from build123d import *

# Parameters (mm, degrees)
SKETCH_1_W          = 365
SKETCH_1_H          = 55
EXTRUDE_1_DEPTH     = 12
SKETCH_2_R          = 10
CUT_EXTRUDE_1_DEPTH = 2
SKETCH_3_W          = 12
SKETCH_3_H          = 55
CUT_EXTRUDE_2_DEPTH = 1.5


with BuildPart() as part:
    # 草图1 → 凸台-拉伸1 (new body)
    with BuildSketch(Plane.XY):
        Rectangle(SKETCH_1_W, SKETCH_1_H)
    extrude(amount=EXTRUDE_1_DEPTH)

    # 草图2 → 切除-拉伸1 (cut)
    with BuildSketch(Plane.XY.offset(12)):
        with Locations((85, 0)):
            Circle(SKETCH_2_R)
        with Locations((-85, 0)):
            Circle(SKETCH_2_R)
    extrude(amount=-CUT_EXTRUDE_1_DEPTH, mode=Mode.SUBTRACT)

    # 草图3 → 切除-拉伸2 (cut)
    with BuildSketch(Plane(origin=(0, 0, 0), x_dir=(-1, 0, 0), z_dir=(0, 0, -1))):
        with Locations((176.5, 0)):
            Rectangle(SKETCH_3_W, SKETCH_3_H)
        with Locations((-176.5, 0)):
            Rectangle(SKETCH_3_W, SKETCH_3_H)
    extrude(amount=-CUT_EXTRUDE_2_DEPTH, mode=Mode.SUBTRACT)


solid = part.part
Source: CAD feature listing. Evaluate the final solid. Frame: model axes, mm. A direction names the side the tool comes from. Coordinates: 2 decimals unless noted, no trailing zeros. Write each loop counter-clockwise with the first axis right and the second up, starting at its lowest first coordinate (ties: lowest second). Pieces come first, ordered by that corner, then holes. Notation, with made-up numbers: M -21,-22.5 L 8,-22.5 A23 cw 8,-7.5 Z; hole C 33,0.25 d11. An arc over 180 degrees is marked long. Use a Markdown table: item, result.
1) Reachability of faces 4 (the flat face through (85, 0, 10)), 5 (the flat face through (-3, -27.5, 6)), 6 (the flat face through (177, 0, 1.5)) from +Z, -Z, +X, -X, +Y, -Y: full face, straight path, thin tool, end or side. Return the list, or none.
Conclusion:
| item | result |
|---|---|
| face 4 | +Z |
| face 5 | +Z, -Z, +X, -X, -Y |
| face 6 | -Z, +X, +Y, -Y |
2) First-contact query: pin 1 Ø10 at (x, y) = (-87, -2) entering from +Z; pin 2 Ø6 at (x, y) = (-178, -8.5) entering from -Z; pin 3 Ø1.2 at (y, z) = (3.5, 0.5) entering from +X. Flat tips, straight axial feed; report the tip coordinate or a pass-through.
Conclusion:
| item | result |
|---|---|
| pin 1 | stops at z = 10 |
| pin 2 | stops at z = 1.5 |
| pin 3 | stops at x = 170.5 |
3) Section A-A, the plane y = 0. Output: boundary loops of the cut face in (x, z).
Conclusion:
| item | result |
|---|---|
| outline | M -182.5,1.5 L -170.5,1.5 L -170.5,0 L 170.5,0 L 170.5,1.5 L 182.5,1.5 L 182.5,12 L 95,12 L 95,10 L 75,10 L 75,12 L -75,12 L -75,10 L -95,10 L -95,12 L -182.5,12 Z |
4) Ray query, L1, parallel to Y at x = -85, z = 11.45; L2, parallel to Z at x = 90, y = -0.5; L3, parallel to X at y = 1.5, z = 1.25. Return the intervals inside material, ascending.
Conclusion:
| item | result |
|---|---|
| L1 | y = -27.5 to -10, 10 to 27.5 |
| L2 | z = 0 to 10 |
| L3 | x = -170.5 to 170.5 |
5) Mould query, pull axis Y, two halves, no side actions, for faces 1 (the flat face through (-176, 0, 1.5)), 2 (the cylindrical face through (75, 0, 11)), 3 (the flat face through (-3, 27.5, 6)). Classes: pulls with the +Y half, pulls with the -Y half, needs draft (parallel to the pull), parting line crosses it, or undercut.
Conclusion:
| item | result |
|---|---|
| face 1 | needs draft |
| face 2 | undercut |
| face 3 | pulls with the +Y half |
6) Section B-B, the plane x = 85. Output: boundary loops of the cut face in (y, z).
Conclusion:
| item | result |
|---|---|
| outline | M -27.5,0 L 27.5,0 L 27.5,12 L 10,12 L 10,10 L -10,10 L -10,12 L -27.5,12 Z |
